Check sheet for the modelled part. Datum: model origin and axes. Units: mm. Give positions to 0.01 mm unless a question says otherwise; leave off trailing zeros. Loops run counter-clockwise (first coordinate to the right, second up) from the corner with the lowest first, then second, coordinate; pieces in that order, holes last. Notation, with made-up numbers: (2.5, 35.5) - (61.5, 35.5) arc R21 cw to (61.5, 49.5) - close; hole circle Ø10 at (-8, 25.25). An arc over 180 degrees is marked (long way). Use one line per item in the form item = value.
from build123d import *

# Parameters (mm, degrees)
MODEL_R             = 2.5
EXTRUDE_1_DEPTH     = 358.5
CUT_EXTRUDE_1_DEPTH = 2420.679144403
HOLE_WIZARD_M6_1_D  = 5


with BuildPart() as part:
    # Model → 凸台-拉伸1 (new, symmetric)
    with BuildSketch(Plane.XY):
        with BuildLine():
            Line((2390.427059452, 419.756797217), (2392.927059452, 419.756797217))
            Line((2392.927059452, 419.756797217), (2392.927059452, 415.406797217))
            Line((2392.927059452, 415.406797217), (2362.927059452, 415.406797217))
            Line((2362.927059452, 415.406797217), (2362.927059452, 419.756797217))
            Line((2362.927059452, 419.756797217), (2365.427059452, 419.756797217))
            Line((2365.427059452, 419.756797217), (2365.427059452, 417.706797217))
            Line((2365.427059452, 417.706797217), (2371.857059452, 417.706797217))
            ThreePointArc((2371.857059452, 417.706797217), (2373.727059452, 422.906797217), (2371.857059452, 428.106797217))
            Line((2371.857059452, 428.106797217), (2365.427059452, 428.106797217))
            Line((2365.427059452, 428.106797217), (2365.427059452, 426.056797217))
            Line((2365.427059452, 426.056797217), (2362.927059452, 426.056797217))
            Line((2362.927059452, 426.056797217), (2362.927059452, 430.406797217))
            Line((2362.927059452, 430.406797217), (2392.927059452, 430.406797217))
            Line((2392.927059452, 430.406797217), (2392.927059452, 426.056797217))
            Line((2392.927059452, 426.056797217), (2390.427059452, 426.056797217))
            Line((2390.427059452, 426.056797217), (2390.427059452, 428.106797217))
            Line((2390.427059452, 428.106797217), (2383.994799144, 428.106797217))
            ThreePointArc((2383.994799144, 428.106797217), (2382.127059452, 422.906797217), (2383.994799144, 417.706797217))
            Line((2383.994799144, 417.706797217), (2390.427059452, 417.706797217))
            Line((2390.427059452, 417.706797217), (2390.427059452, 419.756797217))
        make_face()
        with Locations((2377.927059452, 422.906797217)):
            Circle(MODEL_R, mode=Mode.SUBTRACT)
    extrude(amount=EXTRUDE_1_DEPTH, both=True)

    # 草图1 → 切除-拉伸1 (cut, through all)
    with BuildSketch(Plane(origin=(0, 430.406797217, 0), x_dir=(1, 0, 0), z_dir=(0, 1, 0))):
        Polygon((2362.927059452, 358.5), (2392.927059452, 328.5), (2392.927059452, 358.5), align=None)
        Polygon((2362.927059452, -358.5), (2392.927059452, -328.5), (2392.927059452, -358.5), align=None)
    extrude(amount=-CUT_EXTRUDE_1_DEPTH, mode=Mode.SUBTRACT)

    # M6 螺纹孔1 (through all)
    with Locations(Plane(origin=(0, 430.406797217, 0), x_dir=(1, 0, 0), z_dir=(0, 1, 0))):
        with Locations((2377.927059452, 45), (2377.927059452, -45)):
            Hole(HOLE_WIZARD_M6_1_D / 2)


solid = part.part
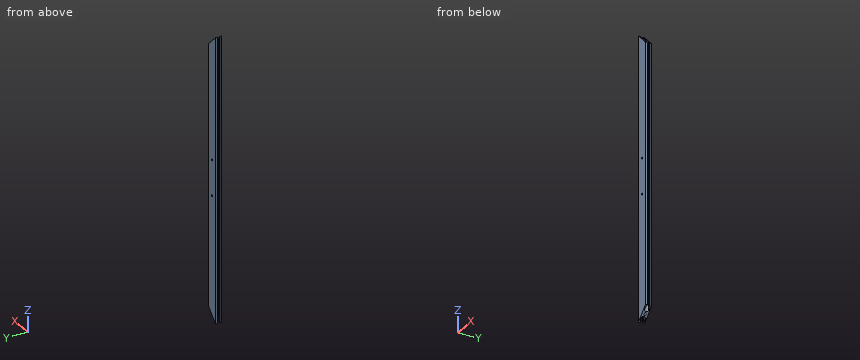
Item 1: Thickness scan on L1, parallel to X at y = 428, z = 317.5; L2, parallel to Z at x = 2380, y = 417; L3, parallel to Y at x = 2365.25, z = 270. Record the ranges inside material, lowest first.
Answer block:
L1 = 2362.93 to 2365.43, 2371.94 to 2383.91, 2390.43 to 2392.93
L2 = -341.43 to -46.4, -43.6 to 43.6, 46.4 to 341.43
L3 = 415.41 to 419.76, 426.06 to 430.41
Item 2: Section check A-A on z = -57.5. Record the boundary of the cut face in (x, y), then the cut area to 3 significant figures.
Answer block:
outline = (2362.93, 415.41) - (2392.93, 415.41) - (2392.93, 419.76) - (2390.43, 419.76) - (2390.43, 417.71) - (2383.99, 417.71) arc R8.17 cw to (2383.99, 428.11) - (2390.43, 428.11) - (2390.43, 426.06) - (2392.93, 426.06) - (2392.93, 430.41) - (2362.93, 430.41) - (2362.93, 426.06) - (2365.43, 426.06) - (2365.43, 428.11) - (2371.86, 428.11) arc R8.16 cw to (2371.86, 417.71) - (2365.43, 417.71) - (2365.43, 419.76) - (2362.93, 419.76) - close; hole circle Ø5 at (2377.93, 422.91)
area = 239 mm2
Item 3: Gauge pin test, flat ends, axial feed: P1, Ø3, axis at x = 2377.93, y = 422.91, coming from the +Z side; P2, Ø6.5, axis at x = 2377.93, z = -45, coming from the +Y side; P3, Ø4, axis at x = 2376, y = 425, coming from the -Z side; P4, Ø8, axis at x = 2377.93, y = 422.91, coming from the +Z side. Record the tip position at first contact, or that the pin passes through.
Answer block:
P1 = through
P2 = 430.41
P3 = -347.43
P4 = 347.5
